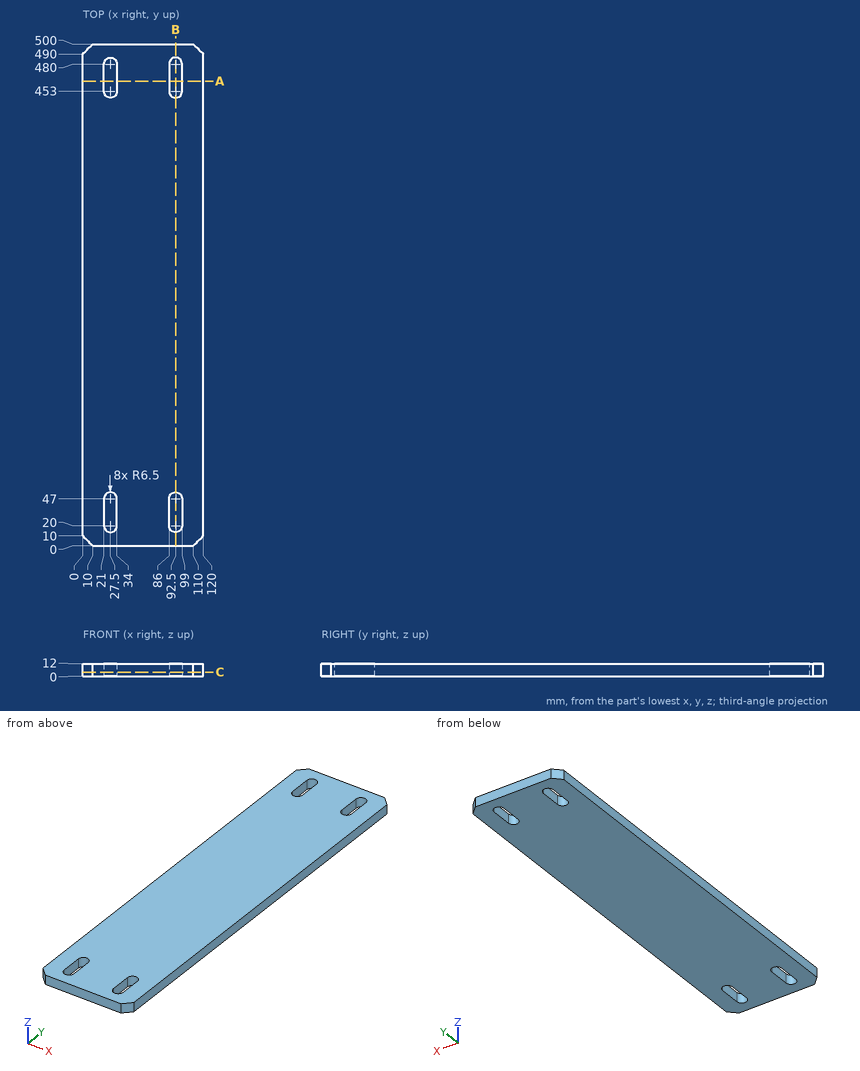
Here's the drawing with two shaded views (mm, measured from the low corner). I have some questions. Give positions to 0.01 mm unless a question says otherwise; leave off trailing zeros. Loops run counter-clockwise (first coordinate to the right, second up) from the corner with the lowest first, then second, coordinate; pieces in that order, holes last. Notation, with made-up numbers: (80.25, -15) - (121.25, -15) arc R30 ccw to (121.25, 18) - close; hole circle Ø10 at (46.5, 50). An arc over 180 degrees is marked (long way). Return JSON: item names as keys, results as strings.
1. I want a section at B-B on x = 92.5. Please give me the cut outline in (y, z).
Output values:
{"outline": "(0, 0) - (13.5, 0) - (13.5, 12) - (0, 12) - close; (53.5, 0) - (446.5, 0) - (446.5, 12) - (53.5, 12) - close; (486.5, 0) - (500, 0) - (500, 12) - (486.5, 12) - close"}
2. If I drill on line 1 (X direction, y = 21, z = 9.5); line 2 (Y direction, x = 23.5, z = 7); line 3 (X direction, y = 53, z = 7.75), over which ranges is the centre line in solid material (lowest first)?
Output values:
{"line 1": "x = 0 to 21, 34 to 86, 99 to 120", "line 2": "y = 0 to 14.88, 52.12 to 447.88, 485.12 to 500", "line 3": "x = 0 to 25, 30 to 90, 95 to 120"}
3. I want a section at A-A on y = 463. Please give me the cut outline in (x, z), and give its area (3 significant figures).
Output values:
{"outline": "(0, 0) - (21, 0) - (21, 12) - (0, 12) - close; (34, 0) - (86, 0) - (86, 12) - (34, 12) - close; (99, 0) - (120, 0) - (120, 12) - (99, 12) - close", "area": "1,130 mm²"}
4. I want a section at C-C on z = 3.75. Please give me the cut outline in (x, y), and give its area (3 significant figures).
Output values:
{"outline": "(0, 10) - (10, 0) - (110, 0) - (120, 10) - (120, 490) - (110, 500) - (10, 500) - (0, 490) - close; hole (21, 20) arc R6.5 ccw to (34, 20) - (34, 47) arc R6.5 ccw to (21, 47) - close; hole (21, 453) arc R6.5 ccw to (34, 453) - (34, 480) arc R6.5 ccw to (21, 480) - close; hole (86, 20) arc R6.5 ccw to (99, 20) - (99, 47) arc R6.5 ccw to (86, 47) - close; hole (86, 453) arc R6.5 ccw to (99, 453) - (99, 480) arc R6.5 ccw to (86, 480) - close", "area": "57,900 mm²"}
